Geometry: final body of the model. Coordinates: model frame, mm. Face numbers are marked on the shaded views. Give positions to 0.01 mm unless a question says otherwise; leave off trailing zeros. Order: outer loops, then holes, each group sorted by start corner. A loop starts at its lowest first (then second) coordinate and runs counter-clockwise, first axis right, second up. Notation, with made-up numbers: (44.5, 83) - (93.5, 83) arc R31 ccw to (93.5, 116) - close; hole circle Ø4 at (52, 45.5). An arc over 180 degrees is marked (long way). Write item = value, one per line. Start each with the question number.
from build123d import *

# Parameters (mm, degrees)
SKETCH1_R           = 10
SKETCH1_R_2         = 6.25
BOSS_EXTRUDE1_DEPTH = 3
CHAMFER1_SIZE       = 0.2


with BuildPart() as part:
    # Sketch1 → Boss-Extrude1 (new body)
    with BuildSketch(Plane.XY):
        Circle(SKETCH1_R)
        Circle(SKETCH1_R_2, mode=Mode.SUBTRACT)
    extrude(amount=BOSS_EXTRUDE1_DEPTH)

    # Chamfer1
    chamfer1_edges = [part.edges().sort_by_distance(p)[0] for p in [
        (-10, 0, 0),
        (-10, 0, 3),
        (-6.25, 0, 0),
        (-6.25, 0, 3),
    ]]
    chamfer(chamfer1_edges, length=CHAMFER1_SIZE)


solid = part.part
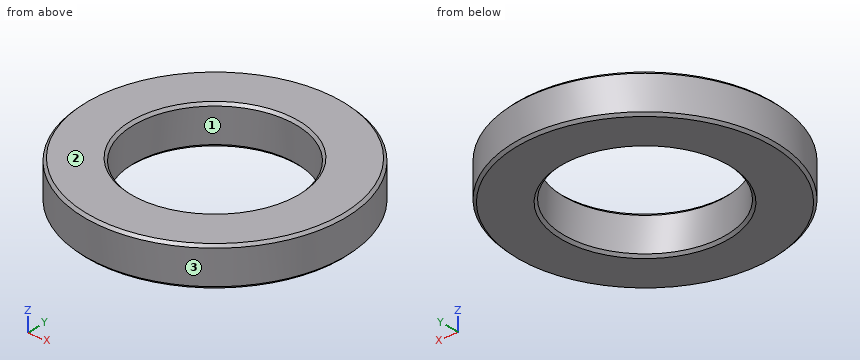
Q1. Section A-A, the plane x = 0. Return the cut outline in (y, z).
Q2. Contact query for flat-ended pins moving along their axis: pin 1 (12 mm diameter, centred on x = 3.5, y = -1.5, fed in from +Z); pin 2 (1 mm diameter, centred on y = 1, z = 1.5, fed in from +X). Output: stop coordinate, or through.
Q3. Section B-B, the plane z = 1.15. Return the cut outline in (x, y).
Q4. Material intervals for line 1 along Y through (x, z) = (0.25, 1.5) (3 decimals); line 2 along X through (y, z) = (4.25, 1.45); line 3 along X through (y, z) = (1.25, 0.4), sorted ascending. Write a range as from..to.
Q5. Pull-direction query (X, two-part tool) for the marked faces 1, 2 and 3; classes: +X half, -X half, draft (parallel to the pull), parting line (faces both ways), or undercut.
The answers:
q1.outline = (-10, 0.2) - (-9.8, 0) - (-6.45, 0) - (-6.25, 0.2) - (-6.25, 2.8) - (-6.45, 3) - (-9.8, 3) - (-10, 2.8) - close; (6.25, 0.2) - (6.45, 0) - (9.8, 0) - (10, 0.2) - (10, 2.8) - (9.8, 3) - (6.45, 3) - (6.25, 2.8) - close
q2.pin_1 = 3
q2.pin_2 = 9.99
q3.outline = circle Ø20 at (0, 0); hole circle Ø12.5 at (0, 0)
q4.line_1 = -9.997..-6.245, 6.245..9.997
q4.line_2 = -9.05..-4.58, 4.58..9.05
q4.line_3 = -9.92..-6.12, 6.12..9.92
q5.face_1 = undercut
q5.face_2 = draft
q5.face_3 = parting line
